The figure shows three views and two pictorial views of one solid part (mm, origin at its lowest corner). Answer the questions. Give positions to 0.01 mm unless a question says otherwise; leave off trailing zeros. Order: outer loops, then holes, each group sorted by start corner. A loop starts at its lowest first (then second) coordinate and runs counter-clockwise, first axis right, second up. Notation, with made-up numbers: (68.25, 73.25) - (124.25, 73.25) arc R13 ccw to (124.25, 89.25) - close; hole circle Ø2 at (10, 49). An arc over 180 degrees is marked (long way). Return JSON: item names as keys, results as strings. Group by question number.
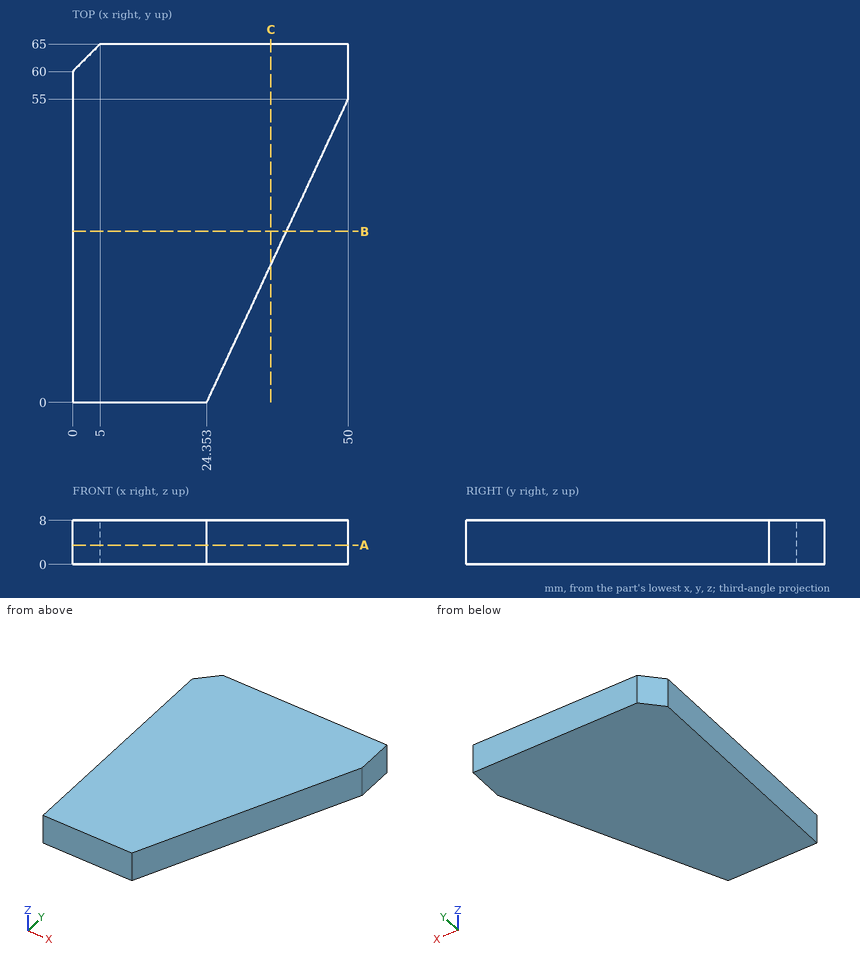
1. Each of these flat-tipped pins is pushed along its axis until it touches: pin 1 (8 mm diameter, centred on x = 44, y = 33.5, fed in from +Z); pin 2 (1.5 mm diameter, centred on y = 35.5, z = 5.5, fed in from +X). Where does it stop, or does it pass through?
2. The part is cut by section B-B (y = 31). Give the vertices of the cut face in (x, z), and give its area (3 significant figures).
3. The part is cut by section A-A (z = 3.5). Give the vertices of the cut face in (x, y), and give its area (3 significant figures).
4. Consider probe 1 along Y at (x, z) = (34, 5.5); probe 2 along X at (y, z) = (49.5, 3.5) (1 decimal); probe 3 along Y at (x, z) = (41.5, 4). Determine where each line is inside the solid, lowest interval first. Write a range as from..to.
5. The part is cut by section C-C (x = 36). Give the vertices of the cut face in (y, z).
Answers:
{
 "1": {"pin 1": "stops at z = 8", "pin 2": "stops at x = 41.26"},
 "2": {"outline": "(0, 0) - (38.81, 0) - (38.81, 8) - (0, 8) - close", "area": "310 mm^2"},
 "3": {"outline": "(0, 0) - (24.35, 0) - (50, 55) - (50, 65) - (5, 65) - (0, 60) - close", "area": "2,530 mm^2"},
 "4": {"probe 1": "y = 20.69..65", "probe 2": "x = 0..47.4", "probe 3": "y = 36.77..65"},
 "5": {"outline": "(24.98, 0) - (65, 0) - (65, 8) - (24.98, 8) - close"}
}
